from build123d import *

# Parameters (mm, degrees)
SKETCH_1_W          = 40
SKETCH_1_H          = 127
EXTRUDE_1_DEPTH     = 2
SKETCH_2_R          = 6.5
CUT_EXTRUDE_1_DEPTH = 3
SKETCH_4_W          = 20
SKETCH_4_H          = 13
CUT_EXTRUDE_4_DEPTH = 10
FILLET_2_R          = 2


with BuildPart() as part:
    # 草图1 → 凸台-拉伸1 (new body)
    with BuildSketch(Plane.XY):
        Rectangle(SKETCH_1_W, SKETCH_1_H)
    extrude(amount=EXTRUDE_1_DEPTH)

    # 草图2 → 切除-拉伸1 (cut)
    with BuildSketch(Plane.XY.offset(2)):
        with Locations((0, 48)):
            Circle(SKETCH_2_R)
        with Locations((0, -48)):
            Circle(SKETCH_2_R)
    extrude(amount=-CUT_EXTRUDE_1_DEPTH, mode=Mode.SUBTRACT)

    # 草图4 → 切除-拉伸4 (cut)
    with BuildSketch(Plane.XY.offset(2)):
        with Locations((10, 48)):
            Rectangle(SKETCH_4_W, SKETCH_4_H)
        with Locations((10, -48)):
            Rectangle(SKETCH_4_W, SKETCH_4_H)
    extrude(amount=-CUT_EXTRUDE_4_DEPTH, mode=Mode.SUBTRACT)

    # 圆角2
    fillet_2_edges = [part.edges().sort_by_distance(p)[0] for p in [
        (20, 54.5, 1),
        (20, 41.5, 1),
        (20, -41.5, 1),
        (20, -54.5, 1),
        (-20, 63.5, 1),
        (20, 63.5, 1),
        (20, -63.5, 1),
        (-20, -63.5, 1),
    ]]
    fillet(fillet_2_edges, radius=FILLET_2_R)


solid = part.part
Build history of the part. All positions in model axes, mm. A direction names the side the tool comes from. Round coordinates to 2 decimals unless told otherwise and drop trailing zeros. Write each loop counter-clockwise with the first axis right and the second up, starting at its lowest first coordinate (ties: lowest second). Pieces come first, ordered by that corner, then holes. Notation, with made-up numbers: (12.25, -39) -> (45.25, -39) arc R9 cw to (45.25, -30) -> close; hole circle Ø5 at (20.5, -2). An arc over 180 degrees is marked (long way). Use one line per item in the form item = value.
Q1. Two-plate mould, pull along Y, no slides. Class faces 3 (the flat face through (9, 41.5, 1)), 4 (the cylindrical face through (19.4, 40.93, 0.99)), 5 (the flat face through (0, 1, 2)), 6 (the cylindrical face through (-19.43, -62.9, 1.01)): released by +Y, released by -Y, zero draft, split by the parting line, or undercut.
Conclusion:
face_3 = undercut
face_4 = undercut
face_5 = zero draft
face_6 = released by -Y
Q2. Band-saw the part on C-C, the plane y = -48. Write the cut outline in (x, z).
Conclusion:
outline = (-20, 0) -> (-6.5, 0) -> (-6.5, 2) -> (-20, 2) -> close
Q3. Band-saw the part on D-D, the plane x = -1.5. Write the cut outline in (y, z).
Conclusion:
outline = (-63.5, 0) -> (-54.32, 0) -> (-54.32, 2) -> (-63.5, 2) -> close; (-41.68, 0) -> (41.68, 0) -> (41.68, 2) -> (-41.68, 2) -> close; (54.32, 0) -> (63.5, 0) -> (63.5, 2) -> (54.32, 2) -> close
Q4. Band-saw the part on A-A, the plane x = 11. Write the cut outline in (y, z), then the cut area to 3 significant figures.
Conclusion:
outline = (-63.5, 0) -> (-54.5, 0) -> (-54.5, 2) -> (-63.5, 2) -> close; (-41.5, 0) -> (41.5, 0) -> (41.5, 2) -> (-41.5, 2) -> close; (54.5, 0) -> (63.5, 0) -> (63.5, 2) -> (54.5, 2) -> close
area = 202 mm²
Q5. Drill centre lines: L1, parallel to Y at x = 11, z = 0.45; L2, parallel to Y at x = -3, z = 1.8; L3, parallel to X at y = -51.5, z = 0.3. Where is each one in solid material? Low to high.
Conclusion:
L1 = -63.5 to -54.5, -41.5 to 41.5, 54.5 to 63.5
L2 = -63.5 to -53.77, -42.23 to 42.23, 53.77 to 63.5
L3 = -20 to -5.48
Q6. Band-saw the part on B-B, the plane z = 1. Write the cut outline in (x, y).
Conclusion:
outline = (-20, -61.5) arc R2 ccw to (-18, -63.5) -> (18, -63.5) arc R2 ccw to (20, -61.5) -> (20, -56.5) arc R2 ccw to (18, -54.5) -> (0, -54.5) arc R6.5 cw to (0, -41.5) -> (18, -41.5) arc R2 ccw to (20, -39.5) -> (20, 39.5) arc R2 ccw to (18, 41.5) -> (0, 41.5) arc R6.5 cw to (0, 54.5) -> (18, 54.5) arc R2 ccw to (20, 56.5) -> (20, 61.5) arc R2 ccw to (18, 63.5) -> (-18, 63.5) arc R2 ccw to (-20, 61.5) -> close
Q7. Tool access for faces 1 (the cylindrical face through (19.43, -40.9, 0.99)), 2 (the flat face through (0, 63.5, 1)): list every direction of +Z, -Z, +X, -X, +Y, -Y with a clear straight run to the whole face (end or side of a thin tool).
Conclusion:
face_1 = +Z, -Z, +X
face_2 = +Z, -Z, +X, -X, +Y
